Input: part model. Units: mm. Frame: model coordinates. A direction names the side the tool comes from. Give positions to 0.01 mm unless a question says otherwise; leave off trailing zeros. Loops run counter-clockwise (first coordinate to the right, second up) from the corner with the lowest first, then second, coordinate; pieces in that order, holes last. Notation, with made-up numbers: M 44,-23.5 L 48,-23.5 A26 ccw 48,15.5 Z; hole C 64,-16 d6. An arc over 180 degrees is marked long. One line per item, written item: value. Start each with the question number.
(1) Section C-C on y = 4.5. Output: boundary loops of the cut face in (x, z).
(2) Section A-A on z = 15.25. Output: boundary loops of the cut face in (x, y), plus the area to 3 significant figures.
(3) Section D-D on z = 2.25. Output: boundary loops of the cut face in (x, y).
(4) Pin query (flat end, axial travel): P1, Ø4, axis at y = 15, z = 16.5, coming from the +X side; P2, Ø4, axis at y = -14.5, z = 22.5, coming from the -X side; P3, Ø1, axis at x = -43, z = 16.5, coming from the +Y side. Return the tip coordinate at first contact, or that it passes through.
(5) Section B-B on x = -7. Output: boundary loops of the cut face in (y, z).
(6) Ray query, line 1 along Z through (x, y) = (-20, -17.5); line 2 along Y through (x, z) = (40.5, 11); line 3 along X through (y, z) = (-15, 10.75). Return the intervals inside material, ascending. Write a range as from..to.
(7) Access query for faces 1 (the cylindrical face through (39.546, 0.274, 1.972)), 2 (the flat face through (-42.249, 15, 16)), 3 (the flat face through (0, 12.483, 2)), 4 (the flat face through (42.249, -15, 16)). Directions: +Z, -Z, +X, -X, +Y, -Y. A direction counts if a zero-diameter tool reaches every point of the face in a straight line with its end or side. Return the directions, or none.
```python
from build123d import *

# Parameters (mm, degrees)
BOSS_EXTRUDE1_DEPTH = 4
BOSS_EXTRUDE2_DEPTH = 25
FILLET1_R           = 2


with BuildPart() as part:
    # Sketch1 → Boss-Extrude1 (new body)
    with BuildSketch(Plane.XY):
        with BuildLine():
            Line((27.065651732, -12.482893197), (-27.188857752, -12.482893197))
            ThreePointArc((-27.188857752, -12.482893197), (-39.671750949, 0), (-27.188857752, 12.482893197))
            Line((-27.188857752, 12.482893197), (27.065651732, 12.482893197))
            ThreePointArc((27.065651732, 12.482893197), (39.548544929, 0), (27.065651732, -12.482893197))
        make_face()
    extrude(amount=BOSS_EXTRUDE1_DEPTH)

    # Sketch2 → Boss-Extrude2 (add)
    with BuildSketch(Plane.XY.offset(4)):
        Polygon((42.249168755, -21.510932303), (-42.249168755, -21.510932303), (-42.249168755, -11.445209118), (-44.167491565, -11.445209118), (-44.167491565, 11.445209118), (-42.249168755, 11.445209118), (-42.249168755, 21.510932303), (42.249168755, 21.510932303), (42.249168755, 11.445209118), (44.167491565, 11.445209118), (44.167491565, -11.445209118), (42.249168755, -11.445209118), align=None)
    extrude(amount=BOSS_EXTRUDE2_DEPTH)

    # Fillet1
    fillet1_edges = [part.edges().sort_by_distance(p)[0] for p in [
        (-42.249168755, 21.510932303, 16.5),
        (-42.249168755, -21.510932303, 16.5),
        (42.249168755, -21.510932303, 16.5),
        (42.249168755, 21.510932303, 16.5),
    ]]
    fillet(fillet1_edges, radius=FILLET1_R)


solid = part.part
```
Output values:
1. outline: M -44.17,4 L -38.83,4 L -38.83,0 L 38.71,0 L 38.71,4 L 44.17,4 L 44.17,29 L -44.17,29 Z
2. outline: M -44.17,-11.45 L -42.25,-11.45 L -42.25,-19.51 A2 ccw -40.25,-21.51 L 40.25,-21.51 A2 ccw 42.25,-19.51 L 42.25,-11.45 L 44.17,-11.45 L 44.17,11.45 L 42.25,11.45 L 42.25,19.51 A2 ccw 40.25,21.51 L -40.25,21.51 A2 ccw -42.25,19.51 L -42.25,11.45 L -44.17,11.45 Z
2. area: 3,720 mm²
3. outline: M -27.19,-12.48 L 27.07,-12.48 A12.48 ccw 27.07,12.48 L -27.19,12.48 A12.48 ccw Z
4. P1: stops at x = 42.25
4. P2: stops at x = -42.25
4. P3: stops at y = 11.45
5. outline: M -21.51,4 L -12.48,4 L -12.48,0 L 12.48,0 L 12.48,4 L 21.51,4 L 21.51,29 L -21.51,29 Z
6. line 1: z = 4..29
6. line 2: y = -21.5..21.5
6. line 3: x = -42.25..42.25
7. face 1: -Z, +X
7. face 2: +Z, -Z, -X, +Y
7. face 3: -Z, +X, -X, +Y
7. face 4: +Z, -Z, +X, -Y
